The figure shows three views and two pictorial views of one solid part (mm, origin at its lowest corner). Answer the questions. A direction names the side the tool comes from. Give positions to 0.01 mm unless a question says otherwise; leave off trailing zeros. Loops run counter-clockwise (first coordinate to the right, second up) from the corner with the lowest first, then second, coordinate; pieces in that order, holes last. Notation, with made-up numbers: M 81,-19 L 128,-19 A19 cw 128,14 Z; hole C 4,-29.5 d10. An arc over 180 degrees is marked long. One line per item, written item: value. Start each with the question number.
Q1. A flat-ended cylindrical pin translates along its axis: pin 1 (5 mm diameter, centred on x = 562, y = 350.5, fed in from -Z). Find the tip coordinate at first contact, or state that the pin passes through.
Q2. A cutting plane is placed at C-C, the plane x = 680. Determine the outline of the cut face in (y, z), and give its area (3 significant figures).
Q3. For the marked faces 1 and 2, determine the directions among +Z, -Z, +X, -X, +Y, -Y from which every point of the face is accessible in a straight line to the end or side of a thin tool.
Q4. Consider L1, parallel to Z at x = 153.5, y = 125.5. Determine where the line is inside the solid, lowest interval first.
Q5. The mould has two halves that part along Z. Classify the marked faces 3, 4 and 5: +Z half, -Z half, draft (parallel to the pull), parting line (faces both ways), or undercut.
Q6. A cutting plane is placed at A-A, the plane z = 411. Determine the outline of the cut face in (x, y).
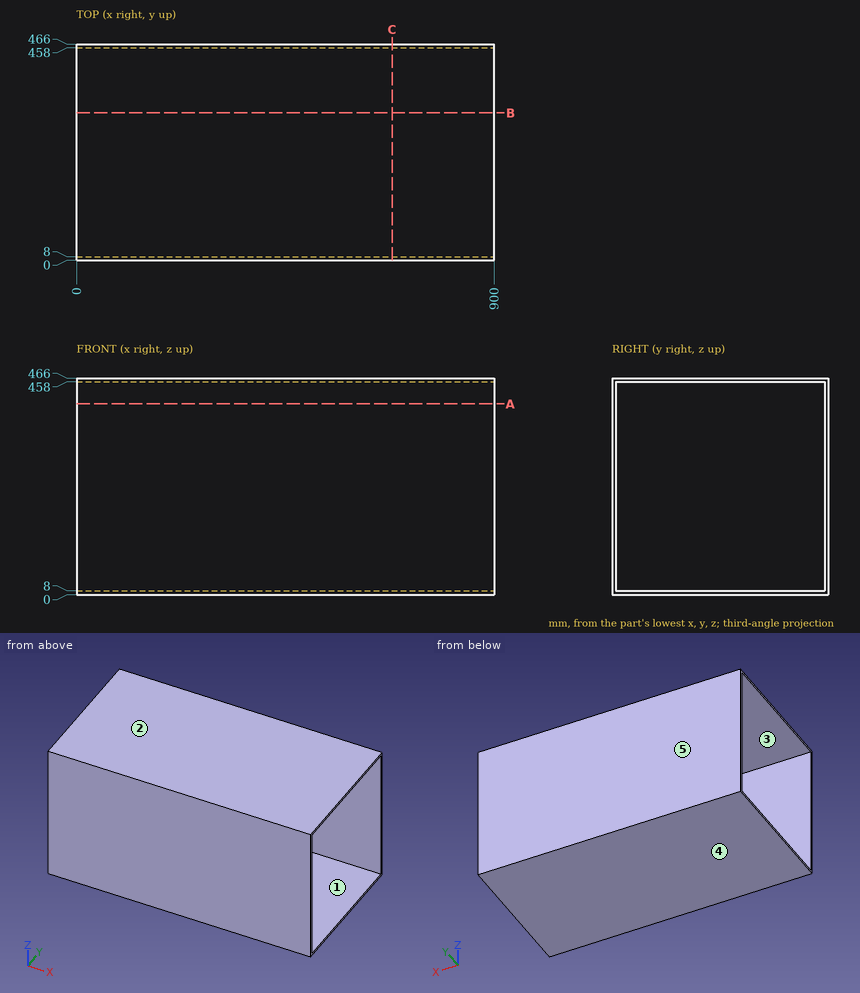
Answer block:
1. pin 1: z = 0
2. outline: M 0,0 L 466,0 L 466,466 L 0,466 Z; hole M 8,8 L 458,8 L 458,458 L 8,458 Z
2. area: 14,700 mm^2
3. face 1: +X, -X
3. face 2: +Z, +X, -X, +Y, -Y
4. L1: 0 to 8, 458 to 466
5. face 3: undercut
5. face 4: -Z half
5. face 5: draft
6. outline: M 0,0 L 900,0 L 900,8 L 0,8 Z; M 0,458 L 900,458 L 900,466 L 0,466 Z
